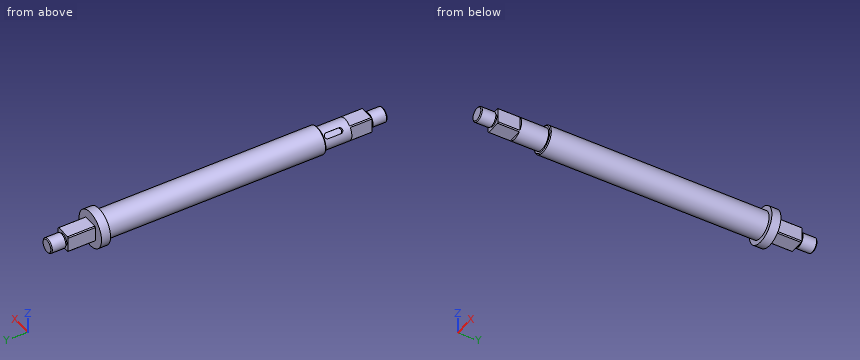
from build123d import *

# Parameters (mm, degrees)
SKETCH_2_OUTSIDE_W   = 117.256
SKETCH_2_OUTSIDE_H   = 117.256
SKETCH_2_OUTSIDE_W_2 = 18
SKETCH_2_OUTSIDE_H_2 = 18
CUT_EXTRUDE_1_DEPTH  = 30
SKETCH_3_OUTSIDE_W   = 117.256
SKETCH_3_OUTSIDE_H   = 117.256
SKETCH_3_OUTSIDE_W_2 = 18
SKETCH_3_OUTSIDE_H_2 = 18
CUT_EXTRUDE_2_DEPTH  = 24
CUT_EXTRUDE_START    = 8.5
CUT_EXTRUDE_3_DEPTH  = 24
CHAMFER_1_SIZE       = 1


with BuildPart() as part:
    # 草图1 → 旋转1 (revolve)
    with BuildSketch(Plane.XY, mode=Mode.PRIVATE) as revolve_1_sk:
        Polygon((0, -186), (0, 186), (-8, 186), (-8, 170), (-6.5, 170), (-6.5, 168), (-12, 168), (-12, 138), (-20, 138), (-20, 128), (-15, 128), (-15, -114), (-12, -114), (-12, -168), (-6.5, -168), (-6.5, -170), (-8, -170), (-8, -186), align=None)
    revolve(revolve_1_sk.sketch.rotate(Axis((0, -186, 0), (0, 1, 0)), 180), axis=Axis((0, -186, 0), (0, 1, 0)))

    # 草图2 outside → 切除-拉伸1 (cut)
    with BuildSketch(Plane(origin=(0, 168, 0), x_dir=(1, 0, 0), z_dir=(0, 1, 0))):
        Rectangle(SKETCH_2_OUTSIDE_W, SKETCH_2_OUTSIDE_H)
        Rectangle(SKETCH_2_OUTSIDE_W_2, SKETCH_2_OUTSIDE_H_2, mode=Mode.SUBTRACT)
    extrude(amount=-CUT_EXTRUDE_1_DEPTH, mode=Mode.SUBTRACT)

    # 草图3 outside → 切除-拉伸2 (cut)
    with BuildSketch(Plane.XZ.offset(168)):
        Rectangle(SKETCH_3_OUTSIDE_W, SKETCH_3_OUTSIDE_H)
        Rectangle(SKETCH_3_OUTSIDE_W_2, SKETCH_3_OUTSIDE_H_2, mode=Mode.SUBTRACT)
    extrude(amount=-CUT_EXTRUDE_2_DEPTH, mode=Mode.SUBTRACT)

    # 草图4 → 切除-拉伸3 (cut)
    with BuildSketch(Plane(origin=(0, 0, 0), x_dir=(0, -1, 0), z_dir=(-0.7071067811865488, 0, 0.7071067811865464)).offset(CUT_EXTRUDE_START)):
        with BuildLine():
            Line((119, 3), (133, 3))
            ThreePointArc((133, 3), (136, 0), (133, -3))
            Line((133, -3), (119, -3))
            ThreePointArc((119, -3), (116, 0), (119, 3))
        make_face()
    extrude(amount=CUT_EXTRUDE_3_DEPTH, mode=Mode.SUBTRACT)

    # 倒角1
    chamfer_1_edges = [part.edges().sort_by_distance(p)[0] for p in [
        (-8, -186, 0),
        (-15, -114, 0),
        (-8, 186, 0),
    ]]
    chamfer(chamfer_1_edges, length=CHAMFER_1_SIZE)


solid = part.part
Verification items for the finished model (mm, model axes). Coordinates: 2 decimals unless noted, no trailing zeros. Write each loop counter-clockwise with the first axis right and the second up, starting at its lowest first coordinate (ties: lowest second). Pieces come first, ordered by that corner, then holes. Notation, with made-up numbers: M -26.75,-24 L 20.25,-24 A14 ccw 20.25,-14 Z; hole C -30,18.25 d4. An arc over 180 degrees is marked long. One line per question, with ' | ' between items.
1) Sectioned sample at B-B on y = -44. Record the cut outline in (x, z).
Solutions:
outline: C 0,0 d30
2) Material ranges on L1, parallel to Y at x = 9.5, z = 6; L2, parallel to Y at x = -1, z = -8; L3, parallel to X at y = -127, z = 5, recorded low to high.
Solutions:
L1: -144 to 138 | L2: -168 to 168 | L3: -10.91 to -9.24, -7.02 to 10.91
3) Depth check by flat-ended pin: pin 1 Ø4 at (y, z) = (21, 3) entering from +X; pin 2 Ø8 at (y, z) = (151.5, 1.5) entering from +X; pin 3 Ø4 at (x, z) = (13.5, 0) entering from -Y. Enter the tip coordinate at first touch or a pass-through.
Solutions:
pin 1: x = 14.97 | pin 2: x = 9 | pin 3: y = -144
4) Sectioned sample at A-A on y = 161. Record the cut outline in (x, z), then the cut area to 3 significant figures.
Solutions:
outline: M -9,-7.94 A12 ccw -7.94,-9 L 7.94,-9 A12 ccw 9,-7.94 L 9,7.94 A12 ccw 7.94,9 L -7.94,9 A12 ccw -9,7.94 Z | area: 322 mm^2
